For this review, use the dimensioned drawing (mm, ordinates from the lowest corner) and the shaded views. A direction names the side the tool comes from. Round coordinates to 2 decimals unless told otherwise and drop trailing zeros. Write each loop counter-clockwise with the first axis right and the second up, starting at its lowest first coordinate (ties: lowest second). Pieces come first, ordered by that corner, then holes. Notation, with made-up numbers: M 74,69.5 L 94,69.5 A24 cw 94,90.5 Z; hole C 65,62 d6. An arc over 180 degrees is marked long. One line per question, with ' | ' between items. Start each with the question number.
Item 1: Add section B-B, the plane y = 29. State the section outline as (x, z) points.
Item 2: Insertion check: pin 1 Ø8 at (x, z) = (39, 15) entering from +Y; pin 2 Ø12 at (x, y) = (24.5, 6.5) entering from +Z; pin 3 Ø7.5 at (y, z) = (18, 21) entering from +X. Each pin has a flat end and moves straight along its axis. Give the tip position at first contact, or say it passes through.
Item 3: Add section A-A, the plane x = 39. State the section outline as (y, z) points.
Item 4: Machinability: for the marked faces 1 and 2, which of the approach directions +Z, -Z, +X, -X, +Y, -Y give a long, thin tool a straight path to every point of the face, cutting with its end or side? Answer none if there is none.
Item 5: Add section C-C, the plane z = 5.5. State the section outline as (x, y) points, and give its area (3 significant figures).
Item 6: For L1, parallel to Y at x = 39, z = 5; L2, parallel to Z at x = 48.5, y = 47; L3, parallel to X at y = 29.5, z = 21, list the stretches that pass through material, from the lowest coordinate up.
Item 7: Add section D-D, the plane y = 7. State the section outline as (x, z) points, and give its area (3 significant figures).
Item 8: Draft analysis for pull direction X (two halves, no side actions). For the marked faces 3, 4 and 5, state which applies: released by +X, released by -X, zero draft, split by the parting line, or undercut.
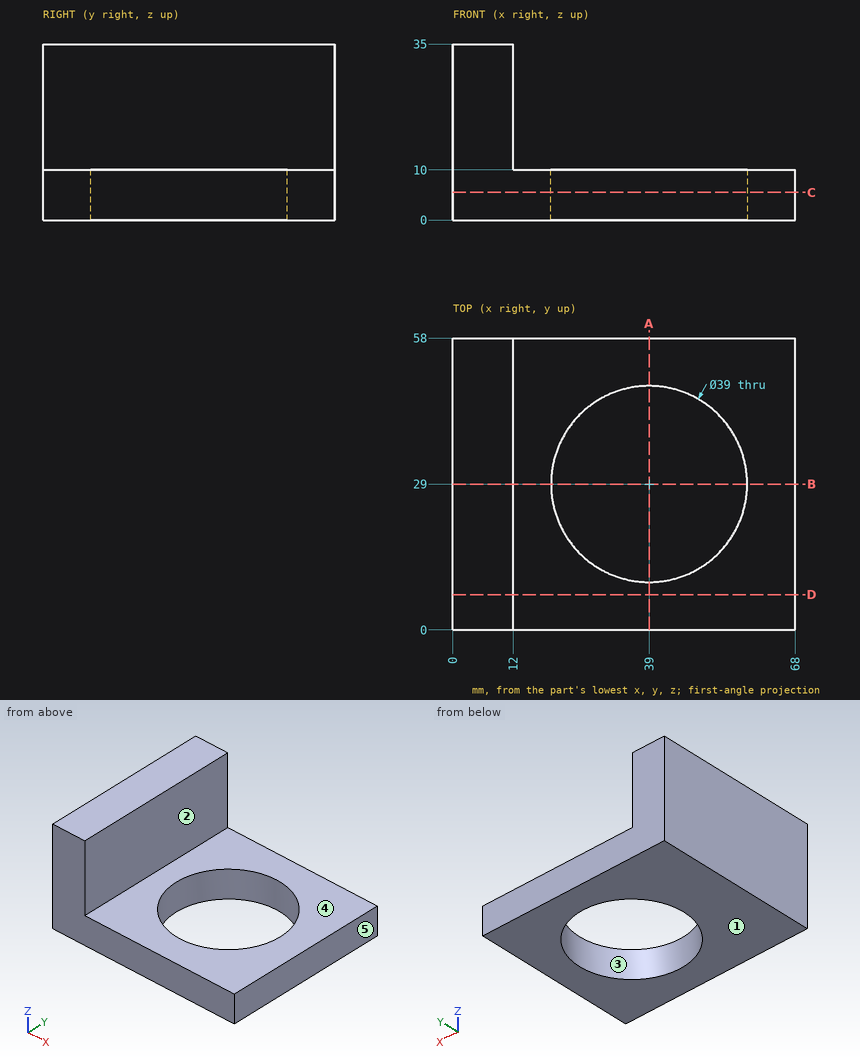
Computed values:
1) outline: M 0,0 L 19.5,0 L 19.5,10 L 12,10 L 12,35 L 0,35 Z; M 58.5,0 L 68,0 L 68,10 L 58.5,10 Z
2) pin 1: passes through | pin 2: stops at z = 10 | pin 3: stops at x = 12
3) outline: M 0,0 L 9.5,0 L 9.5,10 L 0,10 Z; M 48.5,0 L 58,0 L 58,10 L 48.5,10 Z
4) face 1: -Z, +X, -X, +Y, -Y | face 2: +Z, +X, +Y, -Y
5) outline: M 0,0 L 68,0 L 68,58 L 0,58 Z; hole C 39,29 d39 | area: 2,750 mm^2
6) L1: y = 0 to 9.5, 48.5 to 58 | L2: z = 0 to 10 | L3: x = 0 to 12
7) outline: M 0,0 L 68,0 L 68,10 L 12,10 L 12,35 L 0,35 Z | area: 980 mm^2
8) face 3: undercut | face 4: zero draft | face 5: released by +X
